Can you work these out from the model? Positions are in its coordinate system, mm. A direction names the side the tool comes from. Coordinates: 2 decimals unless noted, no trailing zeros. Order: outer loops, then holes, each group sorted by start corner. A loop starts at its lowest first (then second) coordinate and runs counter-clockwise, first axis right, second up. Notation, with made-up numbers: (49, 45.25) -> (79, 45.25) arc R23 ccw to (79, 61.25) -> close; hole circle Ø6 at (-9, 8.25). An arc over 180 degrees is marked (long way). Answer as a JSON object with one key per item and string values. Group by question number.
(1) I want a section at A-A, the plane x = 0. List the corners of the cut face in (y, z) for me, plus the area to 3 significant figures.
(2) Which directions (+Z, -Z, +X, -X, +Y, -Y) give clear straight access to the entire face, cutting with the end or side of a thin tool? Please do faces 4 (the flat face through (4.5, 20, 5)), 5 (the flat face through (0, 40, 5)), 6 (the flat face through (0.1, -35.2, 15)).
(3) I want a section at B-B, the plane y = 29.5. List the corners of the cut face in (x, z) for me, plus the area to 3 significant figures.
(4) If we mould it in two halves opening along Y, with no side actions, what happens to faces 1 (the cylindrical face through (-0.1, 36.5, 5.1)), 2 (the flat face through (-15, -1, 5)), 3 (the flat face through (0, -40, 5))? For each: pulls with the +Y half, pulls with the -Y half, needs draft (parallel to the pull), parting line crosses it, or undercut.
(5) I want a section at D-D, the plane y = -25. List the corners of the cut face in (x, z) for me, plus the area to 3 significant figures.
(6) I need wall thicknesses on line 1 (Z direction, x = 13.75, y = -10); line 2 (Y direction, x = 4, z = 8); line 3 (Y direction, x = -3.25, z = 6.5). Which ranges of each line are inside material? Lowest first, please.
(7) I want a section at C-C, the plane z = 3. List the corners of the cut face in (x, y) for me.
(8) For pin 1 (1 mm diameter, centred on x = 7, y = 31, fed in from +Z); pin 2 (4 mm diameter, centred on x = -3, z = 19.5, fed in from +Y), each with a flat end and sliding along its axis, tell me the tip position at first contact or that it passes through.
from build123d import *

# Parameters (mm, degrees)
SKETCH_1_W          = 30
SKETCH_1_H          = 80
EXTRUDE_1_DEPTH     = 10
SKETCH_2_R          = 12.5
EXTRUDE_2_DEPTH     = 15
CUT_EXTRUDE_START   = -10
SKETCH_3_R          = 12.5
SKETCH_3_R_2        = 10
CUT_EXTRUDE_1_DEPTH = 10
CUT_EXTRUDE_2_DEPTH = 46.276925691
CHAMFER_1_SIZE      = 3


with BuildPart() as part:
    # 草图1 → 凸台-拉伸1 (new body)
    with BuildSketch(Plane.XY):
        Rectangle(SKETCH_1_W, SKETCH_1_H)
    extrude(amount=EXTRUDE_1_DEPTH)

    # 草图2 → 凸台-拉伸2 (add)
    with BuildSketch(Plane.XY.offset(10)):
        with Locations(Location((0, -25, 0), (0, 0, 180))):
            Circle(SKETCH_2_R)
    extrude(amount=EXTRUDE_2_DEPTH)

    # 草图3 → 切除-拉伸1 (cut)
    with BuildSketch(Plane.XY.offset(25).offset(CUT_EXTRUDE_START)):
        with Locations(Location((0, -25, 0), (0, 0, 180))):
            Circle(SKETCH_3_R)
        with Locations((0, -25)):
            Circle(SKETCH_3_R_2, mode=Mode.SUBTRACT)
    extrude(amount=CUT_EXTRUDE_1_DEPTH, mode=Mode.SUBTRACT)

    # 草图4 → 切除-拉伸2 (cut, through all)
    with BuildSketch(Plane.XY.offset(10)):
        with BuildLine():
            Line((4.5, 32), (4.5, 7))
            ThreePointArc((4.5, 7), (0, 2.5), (-4.5, 7))
            Line((-4.5, 7), (-4.5, 32))
            ThreePointArc((-4.5, 32), (0, 36.5), (4.5, 32))
        make_face()
    extrude(amount=-CUT_EXTRUDE_2_DEPTH, mode=Mode.SUBTRACT)

    # 倒角1
    chamfer_1_edges = [part.edges().sort_by_distance(p)[0] for p in [
        (15, -40, 5),
        (-15, -40, 5),
        (-15, 40, 5),
        (15, 40, 5),
    ]]
    chamfer(chamfer_1_edges, length=CHAMFER_1_SIZE)


solid = part.part
Computed values:
{
 "1": {"outline": "(-40, 0) -> (2.5, 0) -> (2.5, 10) -> (-12.5, 10) -> (-12.5, 15) -> (-15, 15) -> (-15, 25) -> (-35, 25) -> (-35, 15) -> (-37.5, 15) -> (-37.5, 10) -> (-40, 10) -> close; (36.5, 0) -> (40, 0) -> (40, 10) -> (36.5, 10) -> close", "area": "785 mm2"},
 "2": {"face 4": "+Z, -Z", "face 5": "+Z, -Z, +X, -X, +Y", "face 6": "+Z"},
 "3": {"outline": "(-15, 0) -> (-4.5, 0) -> (-4.5, 10) -> (-15, 10) -> close; (4.5, 0) -> (15, 0) -> (15, 10) -> (4.5, 10) -> close", "area": "210 mm2"},
 "4": {"face 1": "undercut", "face 2": "needs draft", "face 3": "pulls with the -Y half"},
 "5": {"outline": "(-15, 0) -> (15, 0) -> (15, 10) -> (12.5, 10) -> (12.5, 15) -> (10, 15) -> (10, 25) -> (-10, 25) -> (-10, 15) -> (-12.5, 15) -> (-12.5, 10) -> (-15, 10) -> close", "area": "625 mm2"},
 "6": {"line 1": "z = 0 to 10", "line 2": "y = -40 to 4.94, 34.06 to 40", "line 3": "y = -40 to 3.89, 35.11 to 40"},
 "7": {"outline": "(-15, -37) -> (-12, -40) -> (12, -40) -> (15, -37) -> (15, 37) -> (12, 40) -> (-12, 40) -> (-15, 37) -> close; hole (-4.5, 7) arc R4.5 ccw to (4.5, 7) -> (4.5, 32) arc R4.5 ccw to (-4.5, 32) -> close"},
 "8": {"pin 1": "stops at z = 10", "pin 2": "stops at y = -15.05"}
}
